from build123d import *

# Parameters (mm, degrees)
HEX_HEAD_DEPTH                          = 6
HEAD_TOP_CHAMFER_SKETCH_OUTSIDE_W       = 29.96
HEAD_TOP_CHAMFER_SKETCH_OUTSIDE_H       = 28.722
HEAD_TOP_CHAMFER_SKETCH_OUTSIDE_R       = 4
HEAD_TOP_CHAMFER_45DEG_DEPTH            = 8
HEAD_TOP_CHAMFER_45DEG_DRAFT            = -45
SHANK_SKETCH_R                          = 1.875
SHANK_DEPTH                             = 21.25
HEAD_UNDERSIDE_CHAMFER_SKETCH_OUTSIDE_W = 59.71
HEAD_UNDERSIDE_CHAMFER_SKETCH_OUTSIDE_H = 58.472
HEAD_UNDERSIDE_CHAMFER_SKETCH_OUTSIDE_R = 4
HEAD_UNDERSIDE_CHAMFER_45DEG_DEPTH      = 21.25
HEAD_UNDERSIDE_CHAMFER_45DEG_DRAFT      = -45


with BuildPart() as part:
    # Hex Head Sketch → Hex Head (new body)
    with BuildSketch(Plane(origin=(0, 0, 0), x_dir=(1, 0, 0), z_dir=(0, 1, 0))):
        Polygon((-2.309401077, -4), (2.309401077, -4), (4.618802154, 0), (2.309401077, 4), (-2.309401077, 4), (-4.618802154, 0), align=None)
    extrude(amount=HEX_HEAD_DEPTH)


with BuildPart() as head_top_chamfer_45deg_tool:
    # Head Top Chamfer Sketch outside → Head Top Chamfer 45deg (with draft: the straight prism first)
    with BuildSketch(Plane(origin=(0, 6, 0), x_dir=(1, 0, 0), z_dir=(0, 1, 0))):
        Rectangle(HEAD_TOP_CHAMFER_SKETCH_OUTSIDE_W, HEAD_TOP_CHAMFER_SKETCH_OUTSIDE_H)
        Circle(HEAD_TOP_CHAMFER_SKETCH_OUTSIDE_R, mode=Mode.SUBTRACT)
    extrude(amount=-HEAD_TOP_CHAMFER_45DEG_DEPTH)
    # Head Top Chamfer 45deg: the draft: its side faces are tilted about the plane it starts from
    head_top_chamfer_45deg_sides = [head_top_chamfer_45deg_tool.faces().sort_by_distance(p)[0] for p in [
        (0, 2, 14.361),
        (14.98, 2, 0),
        (0, 2, -14.361),
        (-14.98, 2, 0),
        (-4, 2, 0),
    ]]
    draft(head_top_chamfer_45deg_sides, Plane(origin=(0, 6, 0), x_dir=(1, 0, 0), z_dir=(0, 1, 0)), HEAD_TOP_CHAMFER_45DEG_DRAFT)


with BuildPart() as part_1:
    add(part.part)

    # Head Top Chamfer 45deg: cut by head_top_chamfer_45deg_tool
    add(head_top_chamfer_45deg_tool.part, mode=Mode.SUBTRACT)

    # Shank Sketch → Shank (add)
    with BuildSketch(Plane.XZ):
        with Locations(Location((0, 0, 0), (0, 0, 270))):
            Circle(SHANK_SKETCH_R)
    extrude(amount=SHANK_DEPTH)


with BuildPart() as head_underside_chamfer_45deg_tool:
    # Head Underside Chamfer Sketch outside → Head Underside Chamfer 45deg (with draft: the straight prism first)
    with BuildSketch(Plane.XZ):
        Rectangle(HEAD_UNDERSIDE_CHAMFER_SKETCH_OUTSIDE_W, HEAD_UNDERSIDE_CHAMFER_SKETCH_OUTSIDE_H)
        Circle(HEAD_UNDERSIDE_CHAMFER_SKETCH_OUTSIDE_R, mode=Mode.SUBTRACT)
    extrude(amount=-HEAD_UNDERSIDE_CHAMFER_45DEG_DEPTH)
    # Head Underside Chamfer 45deg: the draft: its side faces are tilted about the plane it starts from
    head_underside_chamfer_45deg_sides = [head_underside_chamfer_45deg_tool.faces().sort_by_distance(p)[0] for p in [
        (0, 10.625, -29.236),
        (29.855, 10.625, 0),
        (0, 10.625, 29.236),
        (-29.855, 10.625, 0),
        (-4, 10.625, 0),
    ]]
    draft(head_underside_chamfer_45deg_sides, Plane.XZ, HEAD_UNDERSIDE_CHAMFER_45DEG_DRAFT)


with BuildPart() as part_2:
    add(part_1.part)

    # Head Underside Chamfer 45deg: cut by head_underside_chamfer_45deg_tool
    add(head_underside_chamfer_45deg_tool.part, mode=Mode.SUBTRACT)


solid = part_2.part
Could you check a few things on this model? Use its own coordinates, in mm. A direction names the side the tool comes from. Give positions to 0.01 mm unless a question says otherwise; leave off trailing zeros. Write each loop counter-clockwise with the first axis right and the second up, starting at its lowest first coordinate (ties: lowest second). Pieces come first, ordered by that corner, then holes. Notation, with made-up numbers: (-32.5, 9) -> (21.5, 9) arc R24 ccw to (21.5, 24) -> close; hole circle Ø11 at (-13.75, 28.5). An arc over 180 degrees is marked (long way). Answer as CSV lines item,"result". Start each with the question number.
(1) Please list where these lines run through material, in increasing order: line 1 (Y direction, x = 3, z = -1.5); line 2 (X direction, y = -5.5, z = 0) (3 decimals); line 3 (Z direction, x = -0.5, y = -3.5).
(2) I'm going to push flat-ended pins straight in: pin 1 Ø4 at (x, y) = (2.5, -3) entering from -Z; pin 2 Ø4 at (x, y) = (3, -5.5) entering from -Z. Where does each tip first touch, or does it pass through?
(3) Which directions (+Z, -Z, +X, -X, +Y, -Y) give clear straight access to the entire face, cutting with the end or side of a thin tool? Please do faces 1 (the face through (0.082, -10.476, 1.873)), 2 (the face through (-4.15, 5.85, -0.01)).
(4) If we section it at B-B, the plane y = 1.75: Write out the boundary of the cut face in (x, z).
(5) If we section it at A-A, the plane y = -9.5: Write out the boundary of the cut face in (x, z) (3 decimals), and give its area (3 significant figures).
Answer list:
1,line 1,"0 to 6"
1,line 2,"-1.875 to 1.875"
1,line 3,"-1.81 to 1.81"
2,pin 1,"z = -1.81"
2,pin 2,"z = -1.59"
3,face 1,"-Y"
3,face 2,"-X, +Y"
4,outline,"(-4.62, 0) -> (-2.31, -4) -> (2.31, -4) -> (4.62, 0) -> (2.31, 4) -> (-2.31, 4) -> close"
5,outline,"circle Ø3.75 at (0, 0)"
5,area,"11.0 mm^2"
